from build123d import *

# Parameters (mm, degrees)
SKETCH1_W             = 44
SKETCH1_H             = 60
BOSS_EXTRUDE1_DEPTH   = 10
CUT_EXTRUDE4_DEPTH    = 15
SKETCH2_W             = 20
SKETCH2_H             = 60
CUT_EXTRUDE1_DEPTH    = 2
M4_TAPPED_HOLE1_D     = 3.3
M4_TAPPED_HOLE1_DEPTH = 10.1
M4_TAPPED_HOLE1_TIP   = 0.991420021
M4_TAPPED_HOLE2_D     = 3.3
M4_TAPPED_HOLE2_DEPTH = 10.1
M4_TAPPED_HOLE2_TIP   = 0.991420021
M3_TAPPED_HOLE2_D     = 2.5
M3_TAPPED_HOLE2_DEPTH = 7.5
M3_TAPPED_HOLE2_TIP   = 0.751075774
CHAMFER3_SIZE         = 0.3
CHAMFER4_SIZE         = 0.5
CUT_EXTRUDE5_DEPTH    = 39.522720569
CHAMFER5_SIZE         = 2
CUT_EXTRUDE6_DEPTH    = 39.522720569


with BuildPart() as part:
    # Sketch1 → Boss-Extrude1 (new body)
    with BuildSketch(Plane.XY):
        Rectangle(SKETCH1_W, SKETCH1_H)
    extrude(amount=BOSS_EXTRUDE1_DEPTH)

    # Sketch13 → Cut-Extrude4 (cut)
    with BuildSketch(Plane(origin=(0, 30, 0), x_dir=(1, 0, 0), z_dir=(0, 1, 0))):
        Polygon((13.25, 0), (14.25, -10), (-14.25, -10), (-13.25, 0), align=None)
    extrude(amount=-CUT_EXTRUDE4_DEPTH, mode=Mode.SUBTRACT)

    # Sketch2 → Cut-Extrude1 (cut)
    with BuildSketch(Plane.XY.offset(10)):
        Rectangle(SKETCH2_W, SKETCH2_H)
    extrude(amount=-CUT_EXTRUDE1_DEPTH, mode=Mode.SUBTRACT)

    # M4 Tapped Hole1
    with Locations(Plane(origin=(0, 30, 0), x_dir=(1, 0, 0), z_dir=(0, 1, 0))):
        with Locations((-17, -5), (17, -5)):
            Hole(M4_TAPPED_HOLE1_D / 2, depth=M4_TAPPED_HOLE1_DEPTH)
            with Locations((0, 0, -(M4_TAPPED_HOLE1_DEPTH + M4_TAPPED_HOLE1_TIP / 2))):  # 118° drill point
                Cone(0, M4_TAPPED_HOLE1_D / 2, M4_TAPPED_HOLE1_TIP, mode=Mode.SUBTRACT)

    # M4 Tapped Hole2
    with Locations(Plane.XY.offset(10)):
        with Locations((-14, -21.5), (14, -21.5), (-14, 3.5), (14, 3.5)):
            Hole(M4_TAPPED_HOLE2_D / 2, depth=M4_TAPPED_HOLE2_DEPTH)
            with Locations((0, 0, -(M4_TAPPED_HOLE2_DEPTH + M4_TAPPED_HOLE2_TIP / 2))):  # 118° drill point
                Cone(0, M4_TAPPED_HOLE2_D / 2, M4_TAPPED_HOLE2_TIP, mode=Mode.SUBTRACT)

    # M3 Tapped Hole2
    with Locations(Plane(origin=(22, 0, 0), x_dir=(0, 0, -1), z_dir=(1, 0, 0))):
        with Locations((-4, -15)):
            Hole(M3_TAPPED_HOLE2_D / 2, depth=M3_TAPPED_HOLE2_DEPTH)
            with Locations((0, 0, -(M3_TAPPED_HOLE2_DEPTH + M3_TAPPED_HOLE2_TIP / 2))):  # 118° drill point
                Cone(0, M3_TAPPED_HOLE2_D / 2, M3_TAPPED_HOLE2_TIP, mode=Mode.SUBTRACT)

    # Chamfer3
    chamfer3_edges = [part.edges().sort_by_distance(p)[0] for p in [
        (-17.625, 30, 0),
        (-18.125, 30, 10),
        (17.625, 30, 0),
        (18.125, 30, 10),
    ]]
    chamfer(chamfer3_edges, length=CHAMFER3_SIZE)

    # Chamfer4
    chamfer4_edges = [part.edges().sort_by_distance(p)[0] for p in [
        (10, -7.5, 10),
        (-10, -7.5, 10),
    ]]
    chamfer(chamfer4_edges, length=CHAMFER4_SIZE)

    # Sketch14 → Cut-Extrude5 (cut, through all)
    with BuildSketch(Plane.XY.offset(10)):
        Polygon((-19, -30), (-19, 3), (-22, 10), (-22, -30), align=None)
        Polygon((19, -30), (19, 3), (22, 10), (22, -30), align=None)
    extrude(amount=-CUT_EXTRUDE5_DEPTH, mode=Mode.SUBTRACT)

    # Chamfer5
    chamfer5_edges = [part.edges().sort_by_distance(p)[0] for p in [
        (-19, -30, 5),
        (19, -30, 5),
    ]]
    chamfer(chamfer5_edges, length=CHAMFER5_SIZE)

    # Sketch15 → Cut-Extrude6 (cut, through all)
    with BuildSketch(Plane(origin=(0, 0, 0), x_dir=(-1, 0, 0), z_dir=(0, 0, -1))):
        with BuildLine():
            Line((-2.5, -5.9), (2.5, -5.9))
            ThreePointArc((2.5, -5.9), (5.1, -8.5), (2.5, -11.1))
            Line((2.5, -11.1), (-2.5, -11.1))
            ThreePointArc((-2.5, -11.1), (-5.1, -8.5), (-2.5, -5.9))
        make_face()
    extrude(amount=-CUT_EXTRUDE6_DEPTH, mode=Mode.SUBTRACT)


solid = part.part
Source: CAD feature listing. Evaluate the final solid. Frame: model axes, mm. A direction names the side the tool comes from. Coordinates: 2 decimals unless noted, no trailing zeros. Loops run counter-clockwise (first coordinate to the right, second up) from the corner with the lowest first, then second, coordinate; pieces in that order, holes last. Notation, with made-up numbers: (-36, -23.75) - (1, -23.75) arc R30 ccw to (1, 10.25) - close; hole circle Ø5 at (-30.5, 1). An arc over 180 degrees is marked (long way). One line per item, written item: value. Start each with the question number.
1. Contact query for flat-ended pins moving along their axis: P1, Ø4, axis at y = -15, z = 4, coming from the +X side; P2, Ø3, axis at x = 7.5, y = -1.5, coming from the +Z side; P3, Ø5, axis at x = -2, z = 6.5, coming from the +Y side. Output: stop coordinate, or through.
2. Set-up query: faces 1 (the flat face through (13.743, 22.605, 4.93)), 2 (the flat face through (-19, -13, 5)), 3 (the flat face through (0, -11.1, 4)), 4 (the flat face through (22, 20, 5)), 5 (the flat face through (-10, -8, 9)). Return all of +Z, -Z, +X, -X, +Y, -Y with unobstructed straight access to the full face (end or side cutting, diameter ignored); none if empty.
3. Section A-A (y = 24). Return the cut outline in (x, z).
4. Section D-D (z = 1.75). Return the cut outline in (x, y) (3 decimals), and give its area (3 significant figures).
5. Mould query, pull axis Y, two halves, no side actions, for faces 6 (the cylindrical face through (5.1, -8.6, 3.9)), 7 (the flat face through (20.5, 6.5, 5.1)), 8 (the flat face through (19, -13, 5)). Classes: pulls with the +Y half, pulls with the -Y half, needs draft (parallel to the pull), parting line crosses it, or undercut.
6. Section C-C (x = 4). Return the cut outline in (y, z), and give its area (3 significant figures).
7. Section B-B (y = -21.5). Return the cut outline in (x, z).
8. Ray query, L1, parallel to X at y = 23.25, z = 5; L2, parallel to Z at x = 15.4, y = -15; L3, parallel to X at y = -26.5, z = 8.5. Return the intervals inside material, ascending.
Verdict:
1. P1: stops at x = 19
1. P2: stops at z = 8
1. P3: stops at y = 15
2. face 1: +Z, +Y
2. face 2: +Z, -Z, -X, -Y
2. face 3: +Z, -Z
2. face 4: +Z, -Z, +X, +Y, -Y
2. face 5: +Z, +Y, -Y
3. outline: (-22, 0) - (-13.25, 0) - (-14.25, 10) - (-22, 10) - close; (13.25, 0) - (22, 0) - (22, 10) - (14.25, 10) - close; hole circle Ø3.3 at (-17, 5); hole circle Ø3.3 at (17, 5)
4. outline: (-22, 10) - (-19, 3) - (-19, -28) - (-17, -30) - (17, -30) - (19, -28) - (19, 3) - (22, 10) - (22, 30) - (13.425, 30) - (13.425, 15) - (-13.425, 15) - (-13.425, 30) - (-22, 30) - close; hole circle Ø3.3 at (-14, -21.5); hole circle Ø3.3 at (-14, 3.5); hole (-2.5, -11.1) - (2.5, -11.1) arc R2.6 ccw to (2.5, -5.9) - (-2.5, -5.9) arc R2.6 ccw to start; hole circle Ø3.3 at (14, -21.5); hole circle Ø3.3 at (14, 3.5)
4. area: 1,930 mm2
5. face 6: undercut
5. face 7: pulls with the -Y half
5. face 8: needs draft
6. outline: (-30, 0) - (-10.62, 0) - (-10.62, 8) - (-30, 8) - close; (-6.38, 0) - (15, 0) - (15, 8) - (-6.38, 8) - close
6. area: 326 mm2
7. outline: (-19, 0) - (-15.65, 0) - (-15.65, 10) - (-19, 10) - close; (-12.35, 0) - (12.35, 0) - (12.35, 10) - (10.5, 10) - (10, 9.5) - (10, 8) - (-10, 8) - (-10, 9.5) - (-10.5, 10) - (-12.35, 10) - close; (15.65, 0) - (19, 0) - (19, 10) - (15.65, 10) - close
8. L1: x = -22 to -18.65, -15.35 to -13.75, 13.75 to 15.35, 18.65 to 22
8. L2: z = 0 to 2.75, 5.25 to 10
8. L3: x = -19 to -10, 10 to 19
